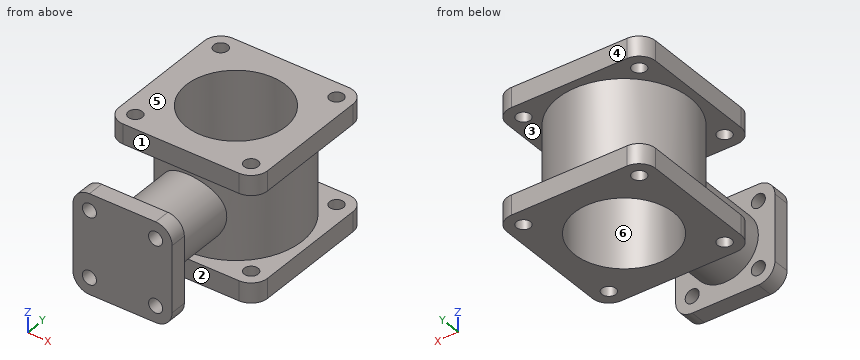
from build123d import *

# Parameters (mm, degrees)
BODY_TUBE_SKETCH_R                 = 40
BODY_TUBE_SKETCH_R_2               = 30
BODY_TUBE_80_DEPTH                 = 52
INLET_FLANGE_SKETCH_W              = 90
INLET_FLANGE_SKETCH_H              = 90
INLET_FLANGE_90X90_DEPTH           = 12
OUTLET_FLANGE_SKETCH_W             = 90
OUTLET_FLANGE_SKETCH_H             = 90
OUTLET_FLANGE_90X90_DEPTH          = 12
FLANGE_BORE_SKETCH_R               = 30
FLANGE_BORE_60_DEPTH               = 100.126182212
OUTLET_FLANGE_CORNER_FILLETS_R10_R = 10
INLET_FLANGE_CORNER_FILLETS_R10_R  = 10
INLET_FLANGE_HOLES_SKETCH_R        = 4.25
INLET_FLANGE_HOLES_4X_8_5_DEPTH    = 12
OUTLET_START                       = -12
OUTLET_FLANGE_HOLES_SKETCH_R       = 4.25
OUTLET_FLANGE_HOLES_4X_8_5_DEPTH   = 12
BRANCH_PIPE_SKETCH_R               = 20
BRANCH_PIPE_40_DEPTH               = 50
MOUNTING_FOOT_SKETCH_W             = 60
MOUNTING_FOOT_SKETCH_H             = 60
MOUNTING_FOOT_60X60_DEPTH          = 10
MOUNTING_FOOT_CORNER_FILLETS_R10_R = 10
MOUNTING_FOOT_HOLES_SKETCH_R       = 4.25
MOUNTING_FOOT_HOLES_4X_8_5_DEPTH   = 10


with BuildPart() as part:
    # Body Tube Sketch → Body Tube Ø80 (new body)
    with BuildSketch(Plane.XY):
        with Locations(Location((0, 0, 0), (0, 0, 180))):
            Circle(BODY_TUBE_SKETCH_R)
        with Locations(Location((0, 0, 0), (0, 0, 180))):
            Circle(BODY_TUBE_SKETCH_R_2, mode=Mode.SUBTRACT)
    extrude(amount=BODY_TUBE_80_DEPTH)

    # Inlet Flange Sketch → Inlet Flange 90x90 (add)
    with BuildSketch(Plane.XY):
        Rectangle(INLET_FLANGE_SKETCH_W, INLET_FLANGE_SKETCH_H)
    extrude(amount=-INLET_FLANGE_90X90_DEPTH)

    # Outlet Flange Sketch → Outlet Flange 90x90 (add)
    with BuildSketch(Plane.XY.offset(52)):
        Rectangle(OUTLET_FLANGE_SKETCH_W, OUTLET_FLANGE_SKETCH_H)
    extrude(amount=OUTLET_FLANGE_90X90_DEPTH)

    # Flange Bore Sketch → Flange Bore Ø60 (cut, through all)
    with BuildSketch(Plane.XY.offset(64)):
        with Locations(Location((0, 0, 0), (0, 0, 180))):
            Circle(FLANGE_BORE_SKETCH_R)
    extrude(amount=-FLANGE_BORE_60_DEPTH, mode=Mode.SUBTRACT)

    # Outlet Flange Corner Fillets R10
    outlet_flange_corner_fillets_r10_edges = [part.edges().sort_by_distance(p)[0] for p in [
        (45, -45, 58),
        (45, 45, 58),
        (-45, 45, 58),
        (-45, -45, 58),
    ]]
    fillet(outlet_flange_corner_fillets_r10_edges, radius=OUTLET_FLANGE_CORNER_FILLETS_R10_R)

    # Inlet Flange Corner Fillets R10
    inlet_flange_corner_fillets_r10_edges = [part.edges().sort_by_distance(p)[0] for p in [
        (-45, -45, -6),
        (-45, 45, -6),
        (45, 45, -6),
        (45, -45, -6),
    ]]
    fillet(inlet_flange_corner_fillets_r10_edges, radius=INLET_FLANGE_CORNER_FILLETS_R10_R)

    # Inlet Flange Holes Sketch → Inlet Flange Holes 4xØ8.5 (cut)
    with BuildSketch(Plane(origin=(0, 0, -12), x_dir=(-1, 0, 0), z_dir=(0, 0, -1))):
        with Locations((-35, 35)):
            Circle(INLET_FLANGE_HOLES_SKETCH_R)
        with Locations((35, 35)):
            Circle(INLET_FLANGE_HOLES_SKETCH_R)
        with Locations((35, -35)):
            Circle(INLET_FLANGE_HOLES_SKETCH_R)
        with Locations((-35, -35)):
            Circle(INLET_FLANGE_HOLES_SKETCH_R)
    extrude(amount=-INLET_FLANGE_HOLES_4X_8_5_DEPTH, mode=Mode.SUBTRACT)

    # Outlet Flange Holes Sketch → Outlet Flange Holes 4xØ8.5 (cut)
    with BuildSketch(Plane.XY.offset(64).offset(OUTLET_START)):
        with Locations(Location((-35, 35, 0), (0, 0, 180))):
            Circle(OUTLET_FLANGE_HOLES_SKETCH_R)
        with Locations(Location((35, 35, 0), (0, 0, 180))):
            Circle(OUTLET_FLANGE_HOLES_SKETCH_R)
        with Locations(Location((35, -35, 0), (0, 0, 180))):
            Circle(OUTLET_FLANGE_HOLES_SKETCH_R)
        with Locations(Location((-35, -35, 0), (0, 0, 180))):
            Circle(OUTLET_FLANGE_HOLES_SKETCH_R)
    extrude(amount=OUTLET_FLANGE_HOLES_4X_8_5_DEPTH, mode=Mode.SUBTRACT)

    # Branch Pipe Sketch → Branch Pipe Ø40 (add)
    with BuildSketch(Plane(origin=(0, -83, 0), x_dir=(1, 0, 0), z_dir=(0, 1, 0))):
        with Locations(Location((0, -26, 0), (0, 0, 90))):
            Circle(BRANCH_PIPE_SKETCH_R)
    extrude(amount=BRANCH_PIPE_40_DEPTH)

    # Mounting Foot Sketch → Mounting Foot 60x60 (add)
    with BuildSketch(Plane(origin=(0, -83, 0), x_dir=(1, 0, 0), z_dir=(0, 1, 0))):
        with Locations((0, -26)):
            Rectangle(MOUNTING_FOOT_SKETCH_W, MOUNTING_FOOT_SKETCH_H)
    extrude(amount=-MOUNTING_FOOT_60X60_DEPTH)

    # Mounting Foot Corner Fillets R10
    mounting_foot_corner_fillets_r10_edges = [part.edges().sort_by_distance(p)[0] for p in [
        (30, -88, -4),
        (30, -88, 56),
        (-30, -88, 56),
        (-30, -88, -4),
    ]]
    fillet(mounting_foot_corner_fillets_r10_edges, radius=MOUNTING_FOOT_CORNER_FILLETS_R10_R)

    # Mounting Foot Holes Sketch → Mounting Foot Holes 4xØ8.5 (cut)
    with BuildSketch(Plane.XZ.offset(93)):
        with Locations(Location((-20, 46, 0), (0, 0, 270))):
            Circle(MOUNTING_FOOT_HOLES_SKETCH_R)
        with Locations(Location((20, 46, 0), (0, 0, 270))):
            Circle(MOUNTING_FOOT_HOLES_SKETCH_R)
        with Locations(Location((20, 6, 0), (0, 0, 270))):
            Circle(MOUNTING_FOOT_HOLES_SKETCH_R)
        with Locations(Location((-20, 6, 0), (0, 0, 270))):
            Circle(MOUNTING_FOOT_HOLES_SKETCH_R)
    extrude(amount=-MOUNTING_FOOT_HOLES_4X_8_5_DEPTH, mode=Mode.SUBTRACT)


solid = part.part
Verification items for the finished model (mm, model axes). Face numbers are marked on the shaded views. A direction names the side the tool comes from. Give positions to 0.01 mm unless a question says otherwise; leave off trailing zeros. Order: outer loops, then holes, each group sorted by start corner. A loop starts at its lowest first (then second) coordinate and runs counter-clockwise, first axis right, second up. Notation, with made-up numbers: M 62,10.25 L 70,10.25 A8 cw 70,17.25 Z; hole C -37.5,-33 d3. An arc over 180 degrees is marked long. Use one line per item in the form item = value. Start each with the question number.
Q1. Scan lines: line 1 along Y through (x, z) = (-35, 56.75); line 2 along Z through (x, y) = (-40, -1.5). Record each from-to range of solid material in increasing order. Write a range as [from, to].
Q2. Go/stop test with flat-tipped pins: pin 1 Ø7 at (x, z) = (-20, 6) entering from -Y; pin 2 Ø3.5 at (x, z) = (17, 58.5) entering from -Y; pin 3 Ø7.5 at (x, y) = (-35, -35) entering from -Z; pin 4 Ø10 at (x, z) = (29, 7.5) entering from +Y. Record where each tip stops, or that it passes through.
Q3. Section check C-C (y = 28). Enter the section's corners in (x, z).
Q4. Section check B-B (x = 0). Enter the section's corners in (y, z).
Q5. Mould release check, pull along Y, two halves, no side actions. Record for the marked faces 4, 5 and 6: +Y half, -Y half, draft (parallel to the pull), parting line (faces both ways), or undercut.
Q6. Section check A-A (z = -2). Enter the section's corners in (x, y), then the cut area to 3 significant figures.
Q7. Access from +Z, -Z, +X, -X, +Y, -Y to the whole of each face (thin tool, end or side, straight path). Record for the marked faces 1, 2 and 3.
Q8. Section check D-D (z = 26). Enter the section's corners in (x, y).
Evaluation:
q1.line_1 = [-45, -39.25], [-30.75, 30.75], [39.25, 45]
q1.line_2 = [-12, 0], [52, 64]
q2.pin_1 = -36.44
q2.pin_2 = -45
q2.pin_3 = through
q2.pin_4 = 32
q3.outline = M -45,-12 L -10.77,-12 L -10.77,64 L -45,64 L -45,52 L -28.57,52 L -28.57,0 L -45,0 Z; M 10.77,-12 L 45,-12 L 45,0 L 28.57,0 L 28.57,52 L 45,52 L 45,64 L 10.77,64 Z
q4.outline = M -93,-4 L -83,-4 L -83,6 L -40,6 L -40,0 L -45,0 L -45,-12 L -30,-12 L -30,64 L -45,64 L -45,52 L -40,52 L -40,46 L -83,46 L -83,56 L -93,56 Z; M 30,-12 L 45,-12 L 45,0 L 40,0 L 40,52 L 45,52 L 45,64 L 30,64 Z
q5.face_4 = +Y half
q5.face_5 = draft
q5.face_6 = undercut
q6.outline = M -45,-35 A10 ccw -35,-45 L 35,-45 A10 ccw 45,-35 L 45,35 A10 ccw 35,45 L -35,45 A10 ccw -45,35 Z; M -26,-93 L 26,-93 L 26,-83 L -26,-83 Z; hole C -35,-35 d8.5; hole C -35,35 d8.5; hole C 0,0 d60; hole C 35,-35 d8.5; hole C 35,35 d8.5
q6.area = 5,480 mm2
q7.face_1 = +Z, +X, -X
q7.face_2 = -Z, +X, -X
q7.face_3 = none
q8.outline = M -30,-93 L 30,-93 L 30,-83 L 20,-83 L 20,-34.64 A40 ccw long -20,-34.64 L -20,-83 L -30,-83 Z; hole C 0,0 d60
